Can you work these out from the model? Positions are in its coordinate system, mm. A direction names the side the tool comes from. Round coordinates to 2 decimals unless told otherwise and drop trailing zeros. Write each loop counter-clockwise with the first axis right and the second up, starting at its lowest first coordinate (ties: lowest second). Pieces come first, ordered by that corner, then holes. Notation, with made-up numbers: M 37.25,87 L 65.25,87 A35 ccw 65.25,123 Z; hole C -39.75,21.5 d3. An arc over 180 degrees is marked long. Answer in a Markdown table with one row per item. Add a question column.
(1) If I drill on probe 1 along X at (y, z) = (5.5, 14); probe 2 along X at (y, z) = (6.5, 3.5); probe 3 along Z at (x, y) = (-204.5, -15.5), over which ranges is the centre line in solid material (lowest first)?
(2) If we mould it in two halves opening along X, with no side actions, what happens to faces 5 (the face through (-293, -3, 8)), 6 (the face through (-217.28, -13.01, 15.08)), 7 (the face through (-108, -32, 10)), 8 (the face through (-292.6, -2.1, 14.6))? For each: released by +X, released by -X, zero draft, split by the parting line, or undercut.
(3) I'm going to push flat-ended pins straight in: pin 1 (5 mm diameter, centred on x = -145, y = -16, fed in from -Z); pin 2 (1 mm diameter, centred on y = -11, z = 6.5, fed in from -X); pin 3 (7 mm diameter, centred on y = -28.5, z = 16, fed in from -X). Where does each tip first touch, or does it pass through?
(4) Suppose I cut it at B-B, the plane y = -21. Write out the boundary of the cut face in (x, z), then the cut area to 3 significant figures.
(5) For faces 1 (the face through (-293, 3, 8)), 2 (the face through (-99, 0, 0)), 3 (the face through (-298, 8.5, 10)), 4 (the face through (-285, 0, 4)), which set-ups out of +Z, -Z, +X, -X, +Y, -Y let a thin tool reach every point of the face, with its end or its side?
(6) Suppose I cut it at C-C, the plane x = -169. Write out the boundary of the cut face in (y, z), then the cut area to 3 significant figures.
(7) Suppose I cut it at D-D, the plane x = -222.5. Write out the boundary of the cut face in (y, z), then the cut area to 3 significant figures.
(8) Suppose I cut it at A-A, the plane z = 4.5. Write out the boundary of the cut face in (x, y), then the cut area to 3 significant figures.
from build123d import *

# Parameters (mm, degrees)
EXTRUDE_1_DEPTH     = 32
SKETCH_2_W          = 87
SKETCH_2_H          = 23.5
CUT_EXTRUDE_1_DEPTH = 22.5
FILLET_1_R          = 15
CUT_EXTRUDE_2_DEPTH = 13
CUT_EXTRUDE_3_REACH = 303.982


with BuildPart() as part:
    # 草图1 → 凸台-拉伸1 (new, symmetric)
    with BuildSketch(Plane(origin=(0, 0, 0), x_dir=(1, 0, 0), z_dir=(0, 1, 0))):
        Polygon((0, 0), (-200, 0), (-200, -9), (-285, -9), (-285, 1.5), (-300, 1.5), (-300, -21), (0, -21), align=None)
    extrude(amount=EXTRUDE_1_DEPTH, both=True)

    # 草图2 → 切除-拉伸1 (cut)
    with BuildSketch(Plane(origin=(0, 0, -1.5), x_dir=(-1, 0, 0), z_dir=(0, 0, -1))):
        with Locations((256.5, -20.25)):
            Rectangle(SKETCH_2_W, SKETCH_2_H)
        with Locations((256.5, 20.25)):
            Rectangle(SKETCH_2_W, SKETCH_2_H)
    extrude(amount=-CUT_EXTRUDE_1_DEPTH, mode=Mode.SUBTRACT)

    # 圆角1
    fillet_1_edges = [part.edges().sort_by_distance(p)[0] for p in [
        (-213, -8.5, 15),
        (-213, 8.5, 15),
    ]]
    fillet(fillet_1_edges, radius=FILLET_1_R)

    # 草图7 → 切除-拉伸2 (cut)
    with BuildSketch(Plane.XY.offset(21)):
        with BuildLine():
            Line((-296.5, 8.5), (-296.5, 6.1))
            ThreePointArc((-296.5, 6.1), (-292.5, 2.1), (-288.5, 6.1))
            Line((-288.5, 6.1), (-288.5, 8.5))
            Line((-288.5, 8.5), (-296.5, 8.5))
        make_face()
    cut_extrude_2 = extrude(amount=-CUT_EXTRUDE_2_DEPTH, mode=Mode.SUBTRACT)

    # 草图8 → 切除-拉伸3 (cut, up to next)
    with BuildSketch(Plane.XY.offset(8), mode=Mode.PRIVATE) as cut_extrude_3_sk1:
        with BuildLine():
            Line((-290.25, 6.1), (-290.25, 8.5))
            Line((-290.25, 8.5), (-294.75, 8.5))
            Line((-294.75, 8.5), (-294.75, 6.1))
            ThreePointArc((-294.75, 6.1), (-292.5, 3.85), (-290.25, 6.1))
        make_face()
    cut_extrude_3_tool1 = extrude(cut_extrude_3_sk1.sketch, amount=-CUT_EXTRUDE_3_REACH, mode=Mode.PRIVATE) & part.part
    cut_extrude_3 = cut_extrude_3_tool1.solids().sort_by_distance((-292.5, 6.386167, 8))[0]
    add(cut_extrude_3, mode=Mode.SUBTRACT)

    # 镜向1: 切除-拉伸2, 切除-拉伸3 across plane
    add(cut_extrude_2.mirror(Plane.ZX), mode=Mode.SUBTRACT)
    add(cut_extrude_3.mirror(Plane.ZX), mode=Mode.SUBTRACT)


solid = part.part
Calculated:
| question | item | result |
|---|---|---|
| 1 | probe 1 | -300 to -296.45, -288.55 to 0 |
| 1 | probe 2 | -300 to -294.75, -290.25 to -285, -200 to 0 |
| 1 | probe 3 | 9 to 21 |
| 2 | face 5 | undercut |
| 2 | face 6 | released by -X |
| 2 | face 7 | zero draft |
| 2 | face 8 | undercut |
| 3 | pin 1 | z = 0 |
| 3 | pin 2 | x = -200 |
| 3 | pin 3 | x = -213 |
| 4 | outline | M -213.21,9 L -200,9 L -200,0 L 0,0 L 0,21 L -213.21,21 Z |
| 4 | area | 4,360 mm² |
| 5 | face 1 | +Z, +Y |
| 5 | face 2 | -Z, +X, +Y, -Y |
| 5 | face 3 | +Z, -Z, -X, +Y |
| 5 | face 4 | -Z, +Y, -Y |
| 6 | outline | M -32,0 L 32,0 L 32,21 L -32,21 Z |
| 6 | area | 1,340 mm² |
| 7 | outline | M -9.54,9 L 9.54,9 L 9.54,21 L -9.54,21 Z |
| 7 | area | 229 mm² |
| 8 | outline | M -300,-8.5 L -294.75,-8.5 L -294.75,-6.1 A2.25 cw -290.25,-6.1 L -290.25,-8.5 L -285,-8.5 L -285,8.5 L -290.25,8.5 L -290.25,6.1 A2.25 cw -294.75,6.1 L -294.75,8.5 L -300,8.5 Z; M -200,-32 L 0,-32 L 0,32 L -200,32 Z |
| 8 | area | 13,000 mm² |
